Can you work these out from the drawing? Everything is in mm from the part's minimum corner. Give positions to 0.01 mm unless a question says otherwise; leave off trailing zeros. Write each loop counter-clockwise with the first axis right and the second up, starting at its lowest first coordinate (ties: lowest second). Pieces come first, ordered by that corner, then holes. Notation, with made-up numbers: (-29.5, 1.5) - (-17.5, 1.5) arc R12 cw to (-17.5, 17.5) - close; hole circle Ø5 at (-29, 3.5). An arc over 180 degrees is marked (long way). Use a Markdown table: item, result.
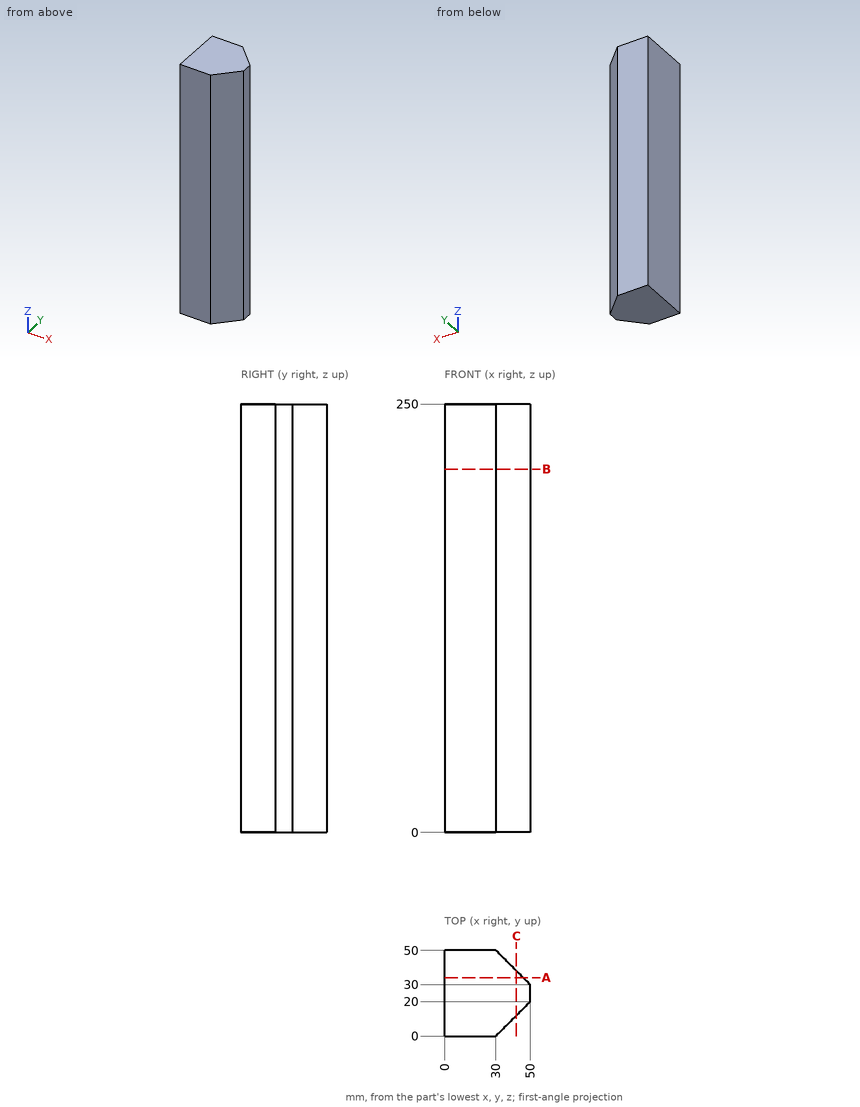
Item 1: If we section it at A-A, the plane y = 34: Write out the boundary of the cut face in (x, z), plus the area to 3 significant figures.
Values:
| item | result |
|---|---|
| outline | (0, 0) - (46, 0) - (46, 250) - (0, 250) - close |
| area | 11,500 mm2 |
Item 2: If we section it at C-C, the plane x = 42: Write out the boundary of the cut face in (y, z).
Values:
| item | result |
|---|---|
| outline | (12, 0) - (38, 0) - (38, 250) - (12, 250) - close |
Item 3: I need wall thicknesses on line 1 along Y through (x, z) = (46, 120.5); line 2 along X through (y, z) = (33, 144); line 3 along X through (y, z) = (46.5, 161). Which ranges of each line are inside material? Lowest first, please. Write a range as [from, to].
Values:
| item | result |
|---|---|
| line 1 | y = [16, 34] |
| line 2 | x = [0, 47] |
| line 3 | x = [0, 33.5] |
Item 4: If we section it at B-B, the plane z = 212: Write out the boundary of the cut face in (x, y), plus the area to 3 significant figures.
Values:
| item | result |
|---|---|
| outline | (0, 0) - (30, 0) - (50, 20) - (50, 30) - (30, 50) - (0, 50) - close |
| area | 2,100 mm2 |
Item 5: Will this pin go through, and if not, where does the flat tip stop? pin 1 Ø3 at (x, z) = (34.5, 74) entering from +Y.
Values:
| item | result |
|---|---|
| pin 1 | stops at y = 47 |
